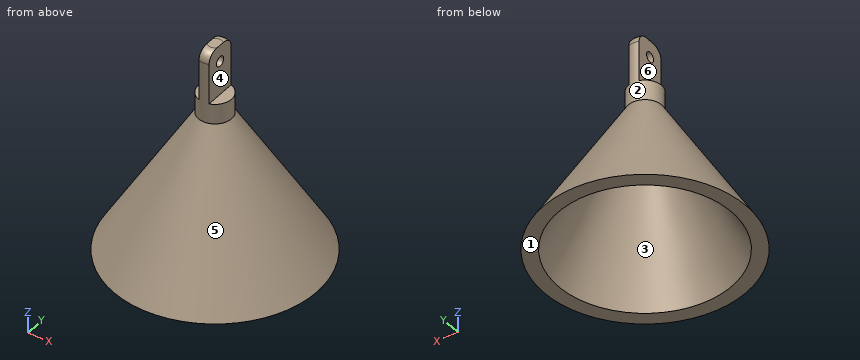
from build123d import *

# Parameters (mm, degrees)
SKETCH2_W          = 22.958469665
SKETCH2_H          = 42.577525561
CUT_EXTRUDE1_DEPTH = 50
SKETCH3_R          = 5
CUT_EXTRUDE2_DEPTH = 50
FILLET1_R          = 10


with BuildPart() as part:
    # Sketch1 → Revolve1 (revolve)
    with BuildSketch(Plane(origin=(0, 0, 0), x_dir=(1, 0, 0), z_dir=(0, 1, 0)), mode=Mode.PRIVATE) as revolve1_sk:
        Polygon((0, 0), (16.40283031, 0), (16.40283031, 69.874110237), (100.714201253, 209.625997087), (8.201415155, 209.625997087), (0, 209.625997087), align=None)
    revolve(revolve1_sk.sketch.rotate(Axis((0, 0, 0), (0, 0, -1)), 180), axis=Axis((0, 0, 0), (0, 0, -1)))

    # Sketch2 → Cut-Extrude1 (cut)
    with BuildSketch(Plane.XY):
        with Locations((-16.479234833, -2.283064826)):
            Rectangle(SKETCH2_W, SKETCH2_H)
        with Locations((16.479234833, -2.283064826)):
            Rectangle(SKETCH2_W, SKETCH2_H)
    extrude(amount=-CUT_EXTRUDE1_DEPTH, mode=Mode.SUBTRACT)

    # Sketch3 → Cut-Extrude2 (cut)
    with BuildSketch(Plane(origin=(5, 0, 0), x_dir=(0, 0, -1), z_dir=(1, 0, 0))):
        with Locations(Location((16.498374342, 0, 0), (0, 0, 90))):
            Circle(SKETCH3_R)
    extrude(amount=-CUT_EXTRUDE2_DEPTH, mode=Mode.SUBTRACT)

    # Fillet1
    fillet1_edges = [part.edges().sort_by_distance(p)[0] for p in [
        (0, -16.40283031, 0),
        (0, 16.40283031, 0),
    ]]
    fillet(fillet1_edges, radius=FILLET1_R)

    # Sketch4 → Cut-Revolve1 (revolve, cut)
    with BuildSketch(Plane(origin=(0, 0, 0), x_dir=(0, 0, -1), z_dir=(1, 0, 0)), mode=Mode.PRIVATE) as cut_revolve1_sk:
        Polygon((77.000967597, 14.066660466), (233.165313112, 99.181638622), (233.165313112, 0), (77.000967597, 0), align=None)
    revolve(cut_revolve1_sk.sketch.rotate(Axis((0, 0, -233.165313112), (0, 0, 1)), 197.747662393), axis=Axis((0, 0, -233.165313112), (0, 0, 1)), mode=Mode.SUBTRACT)


solid = part.part
Build history of the part. All positions in model axes, mm. Face numbers are marked on the shaded views. A direction names the side the tool comes from. Give positions to 0.01 mm unless a question says otherwise; leave off trailing zeros. Write each loop counter-clockwise with the first axis right and the second up, starting at its lowest first coordinate (ties: lowest second). Pieces come first, ordered by that corner, then holes. Notation, with made-up numbers: (57, 84) - (101, 84) arc R31 cw to (101, 114) - close; hole circle Ø9 at (-4, -1.75). An arc over 180 degrees is marked (long way). Use one line per item in the form item = value. Start each with the question number.
1. Band-saw the part on B-B on z = -29.5. Write the cut outline in (x, y), plus the area to 3 significant figures.
2. Two-plate mould, pull along Y, no slides. Class the marked faces 1, 2 and 3: released by +Y, released by -Y, zero draft, split by the parting line, or undercut.
3. 3-axis set-ups, long thin cutter, end or side, ignore diameter. For the marked faces 4, 5 and 6: which of +Z, -Z, +X, -X, +Y, -Y reach the whole face in a straight line?
4. Band-saw the part on A-A on y = 0. Write the cut outline in (x, z), plus the area to 3 significant figures.
5. Probe line 1 (Z direction, x = -3, y = 0); line 2 (X direction, y = -41.5, z = -163); line 3 (X direction, y = 23.5, z = -107). List the from-to ranges inside material, lowest first. Write a range as [from, to].
6. Drop flat-ended pins along their axis: pin 1 Ø8 at (y, z) = (-16, -170.5) entering from +X; pin 2 Ø25 at (y, z) = (1, -34.5) entering from +X; pin 3 Ø25 at (y, z) = (7.5, -25.5) entering from -X. Give the stop position or say it passes through.
Conclusion:
q1.outline = (-5, -15.62) arc R16.4 ccw to (5, -15.62) - (5, 15.62) arc R16.4 ccw to (-5, 15.62) - close
q1.area = 323 mm²
q2.face_1 = zero draft
q2.face_2 = split by the parting line
q2.face_3 = undercut
q3.face_4 = +Z, +X, +Y, -Y
q3.face_5 = +Z
q3.face_6 = +Z, -X, +Y, -Y
q4.outline = (-100.71, -209.63) - (-86.35, -209.63) - (-14.07, -77) - (14.07, -77) - (86.35, -209.63) - (100.71, -209.63) - (16.4, -69.87) - (16.4, -50) - (5, -50) - (5, -21.5) - (-5, -21.5) - (-5, -50) - (-16.4, -50) - (-16.4, -69.87) - close; (-5, -11.5) - (5, -11.5) - (5, 0) - (-5, 0) - close
q4.area = 4,100 mm²
q5.line_1 = [-77, -21.5], [-11.5, 0]
q5.line_2 = [-59.55, -44.62], [44.62, 59.55]
q5.line_3 = [-30.87, -19.31], [19.31, 30.87]
q6.pin_1 = 78.02
q6.pin_2 = 5
q6.pin_3 = -5
